from build123d import *

# Parameters (mm, degrees)
BOSS_EXTRUDE1_DEPTH = 10


with BuildPart() as part:
    # Sketch1 → Boss-Extrude1 (new body)
    with BuildSketch(Plane.XY):
        with BuildLine():
            ThreePointArc((893.221093202, 341.53568212), (914.498906919, 369.426423756), (894.770629974, 398.433904074))
            Line((894.770629974, 398.433904074), (746.5, 452.4))
            Line((746.5, 452.4), (746.5, 480.1))
            ThreePointArc((746.5, 480.1), (924.530143798, 456.633232126), (1101.599381764, 426.768432422))
            Line((1101.599381764, 426.768432422), (1102.628920146, 425.298099233))
            ThreePointArc((1102.628920146, 425.298099233), (1071.5, 365.5), (1102.628920146, 305.701900767))
            Line((1102.628920146, 305.701900767), (1098.632098759, 299.99384827))
            ThreePointArc((1098.632098759, 299.99384827), (593.965714202, 137.948571105), (109.234583042, -76.486878479))
            Line((109.234583042, -76.486878479), (104.851461669, -73.417783853))
            ThreePointArc((104.851461669, -73.417783853), (126.422272258, -20.035195957), (122.413865115, 37.401144736))
            ThreePointArc((122.413865115, 37.401144736), (501.640075089, 205.12460213), (893.221093202, 341.53568212))
        make_face()
    extrude(amount=BOSS_EXTRUDE1_DEPTH)


solid = part.part
Verification items for the finished model (mm, model axes). A direction names the side the tool comes from. Give positions to 0.01 mm unless a question says otherwise; leave off trailing zeros. Order: outer loops, then holes, each group sorted by start corner. A loop starts at its lowest first (then second) coordinate and runs counter-clockwise, first axis right, second up. Notation, with made-up numbers: M 43,-25 L 64,-25 A9 ccw 64,-11 Z; hole C -33,38.5 d1. An arc over 180 degrees is marked long. Use one line per item in the form item = value. Start each with the question number.
Q1. Section check B-B (z = 7). Enter the section's corners in (x, y) (3 decimals), then the cut area to 3 significant figures.
Q2. Section check C-C (y = -3.5). Enter the section's corners in (x, z).
Q3. Scan lines: line 1 along Y through (x, z) = (768.5, 9); line 2 along Y through (x, z) = (808.5, 1.75); line 3 along X through (y, z) = (10, 6.25). Record each from-to range of solid material in increasing order. Write a range as [from, to].
Q4. Access from +Z, -Z, +X, -X, +Y, -Y to the whole of each face (thin tool, end or side, straight path). Record for faces 4 (the flat face through (643, 203, 0)), 5 (the cylindrical face through (496.24, 202.99, 4.93)).
Q5. Mould release check, pull along Y, two halves, no side actions. Record for faces 1 (the cylindrical face through (1071.507, 366.481, 4.93)), 2 (the flat face through (643, 203, 10)), 3 (the cylindrical face through (922.044, 457.006, 4.93)): +Y half, -Y half, draft (parallel to the pull), parting line (faces both ways), or undercut.
Q6. Go/stop test with flat-tipped pins: pin 1 Ø5 at (y, z) = (461, 6.5) entering from -X; pin 2 Ø2 at (x, z) = (349.5, 7.5) entering from +Y; pin 3 Ø1 at (x, z) = (441.5, 4) entering from -Y. Record where each tip stops, or that it passes through.
Q7. Section check D-D (x = 880). Enter the section's corners in (y, z).
Q8. Section check A-A (x = 775.5). Enter the section's corners in (y, z), then the cut area to 3 significant figures.
Evaluation:
q1.outline = M 104.851,-73.418 L 109.235,-76.487 A5012 cw 1098.632,299.994 L 1102.629,305.702 A73 cw 1102.629,425.298 L 1101.599,426.768 A4984 ccw 746.5,480.1 L 746.5,452.4 L 894.771,398.434 A30 cw 893.221,341.536 A5108 ccw 122.414,37.401 A128 cw Z
q1.area = 119,000 mm2
q2.outline = M 127.95,0 L 259.27,0 L 259.27,10 L 127.95,10 Z
q3.line_1 = [200.69, 301.94], [444.39, 477.55]
q3.line_2 = [214.05, 315.02], [429.83, 472.67]
q3.line_3 = [127.61, 288.48]
q4.face_4 = -Z, +X, -X, +Y, -Y
q4.face_5 = +Z, -Z, -X
q5.face_1 = undercut
q5.face_2 = draft
q5.face_3 = +Y half
q6.pin_1 = 746.5
q6.pin_2 = 142.68
q6.pin_3 = 76.85
q7.outline = M 237.01,0 L 337.5,0 L 337.5,10 L 237.01,10 Z; M 403.81,0 L 463.12,0 L 463.12,10 L 403.81,10 Z
q8.outline = M 203.06,0 L 304.25,0 L 304.25,10 L 203.06,10 Z; M 441.84,0 L 476.72,0 L 476.72,10 L 441.84,10 Z
q8.area = 1,360 mm2
